Work out the finished part from the listing and answer in its coordinate system (mm). A direction names the side the tool comes from. Round coordinates to 2 decimals unless told otherwise and drop trailing zeros. Write each loop counter-clockwise with the first axis right and the second up, starting at its lowest first coordinate (ties: lowest second). Pieces come first, ordered by that corner, then holes.
from build123d import *

# Parameters (mm, degrees)
SKETCH1_R           = 19
SKETCH1_R_2         = 8.25
BOSS_EXTRUDE1_DEPTH = 2.5
SKETCH2_R           = 10
BOSS_EXTRUDE2_DEPTH = 10
SKETCH3_R           = 1.75
CUT_EXTRUDE1_DEPTH  = 10
CHAMFER1_SIZE       = 1
M6_TAPPED_HOLE1_D   = 5


with BuildPart() as part:
    # Sketch1 → Boss-Extrude1 (new body)
    with BuildSketch(Plane.XY):
        Circle(SKETCH1_R)
        Circle(SKETCH1_R_2, mode=Mode.SUBTRACT)
    extrude(amount=BOSS_EXTRUDE1_DEPTH)

    # Sketch2 → Boss-Extrude2 (add)
    with BuildSketch(Plane.XY.offset(2.5)):
        Circle(SKETCH2_R)
    extrude(amount=BOSS_EXTRUDE2_DEPTH)

    # Sketch3 → Cut-Extrude1 (cut)
    with BuildSketch(Plane.XY.offset(2.5)):
        with Locations((15, 0)):
            Circle(SKETCH3_R)
        with Locations((0, 15)):
            Circle(SKETCH3_R)
        with Locations((-15, 0)):
            Circle(SKETCH3_R)
        with Locations((0, -15)):
            Circle(SKETCH3_R)
    extrude(amount=-CUT_EXTRUDE1_DEPTH, mode=Mode.SUBTRACT)

    # Chamfer1
    chamfer1_edges = [part.edges().sort_by_distance(p)[0] for p in [
        (-10, 0, 12.5),
    ]]
    chamfer(chamfer1_edges, length=CHAMFER1_SIZE)

    # M6 Tapped Hole1 (through all)
    with Locations(Plane.XY.offset(12.5)):
        with Locations((0, 0)):
            Hole(M6_TAPPED_HOLE1_D / 2)


solid = part.part
Q1. A tool of negligible diameter and unlimited length cuts with its end or side. For faces 1 (the face through (8, -8, 2.5)), 2 (the face through (7.62, -3.16, 1.23)), 3 (the face through (0.54, -2.44, 7.43)), from which of +Z, -Z, +X, -X, +Y, -Y can it reach the whole face along a straight path? Write none if from no direction.
Q2. Given pin 1 (3 mm diameter, centred on y = 8, z = 9, fed in from -X); pin 2 (8 mm diameter, centred on x = -1, y = 2.5, fed in from -Z); pin 3 (5 mm diameter, centred on x = -9.5, z = 7, fed in from +Y), each flat-ended and moving along its own axis, determine where each tip first touches the part or whether it passes through.
Q3. Find section A-A (y = 0). Determine the outline of the cut face in (x, z), plus the area to 3 significant figures.
Q4. The mould has two halves that part along Y. Classify faces 4 (the face through (-0.228, -13.265, 1.268)), 5 (the face through (-9, 0, 0)), 6 (the face through (-2.17, -9.76, 6.94)): +Y half, -Y half, draft (parallel to the pull), parting line (faces both ways), or undercut.
Q5. Find the intervals of material crossed by L1, parallel to Y at x = 0, z = 1.65; L2, parallel to Z at x = -4, y = -10; L3, parallel to Z at x = -4, y = -5.5, in increasing order.
Q6. Find section C-C (z = 3.5). Determine the outline of the cut face in (x, y), plus the area to 3 significant figures.
Q7. Find section B-B (y = 15). Determine the outline of the cut face in (x, z), plus the area to 3 significant figures.
Report:
1. face 1: +Z
1. face 2: -Z
1. face 3: +Z, -Z
2. pin 1: stops at x = -7.6
2. pin 2: stops at z = 2.5
2. pin 3: stops at y = 7.14
3. outline: (-19, 0) - (-16.75, 0) - (-16.75, 2.5) - (-19, 2.5) - close; (-13.25, 0) - (-8.25, 0) - (-8.25, 2.5) - (-2.5, 2.5) - (-2.5, 12.5) - (-9, 12.5) - (-10, 11.5) - (-10, 2.5) - (-13.25, 2.5) - close; (2.5, 2.5) - (8.25, 2.5) - (8.25, 0) - (13.25, 0) - (13.25, 2.5) - (10, 2.5) - (10, 11.5) - (9, 12.5) - (2.5, 12.5) - close; (16.75, 0) - (19, 0) - (19, 2.5) - (16.75, 2.5) - close
3. area: 185 mm2
4. face 4: undercut
4. face 5: draft
4. face 6: parting line
5. L1: y = -19 to -16.75, -13.25 to -8.25, 8.25 to 13.25, 16.75 to 19
5. L2: z = 0 to 2.5
5. L3: z = 2.5 to 12.5
6. outline: circle Ø20 at (0, 0); hole circle Ø5 at (0, 0)
6. area: 295 mm2
7. outline: (-11.66, 0) - (-1.75, 0) - (-1.75, 2.5) - (-11.66, 2.5) - close; (1.75, 0) - (11.66, 0) - (11.66, 2.5) - (1.75, 2.5) - close
7. area: 49.6 mm2
